Geometry: see drawing. Coordinates: mm, zero at the bounding-box minimum. A direction names the side the tool comes from. Coordinates: 2 decimals unless noted, no trailing zeros. Loops run counter-clockwise (first coordinate to the right, second up) from the corner with the lowest first, then second, coordinate; pieces in that order, holes last.
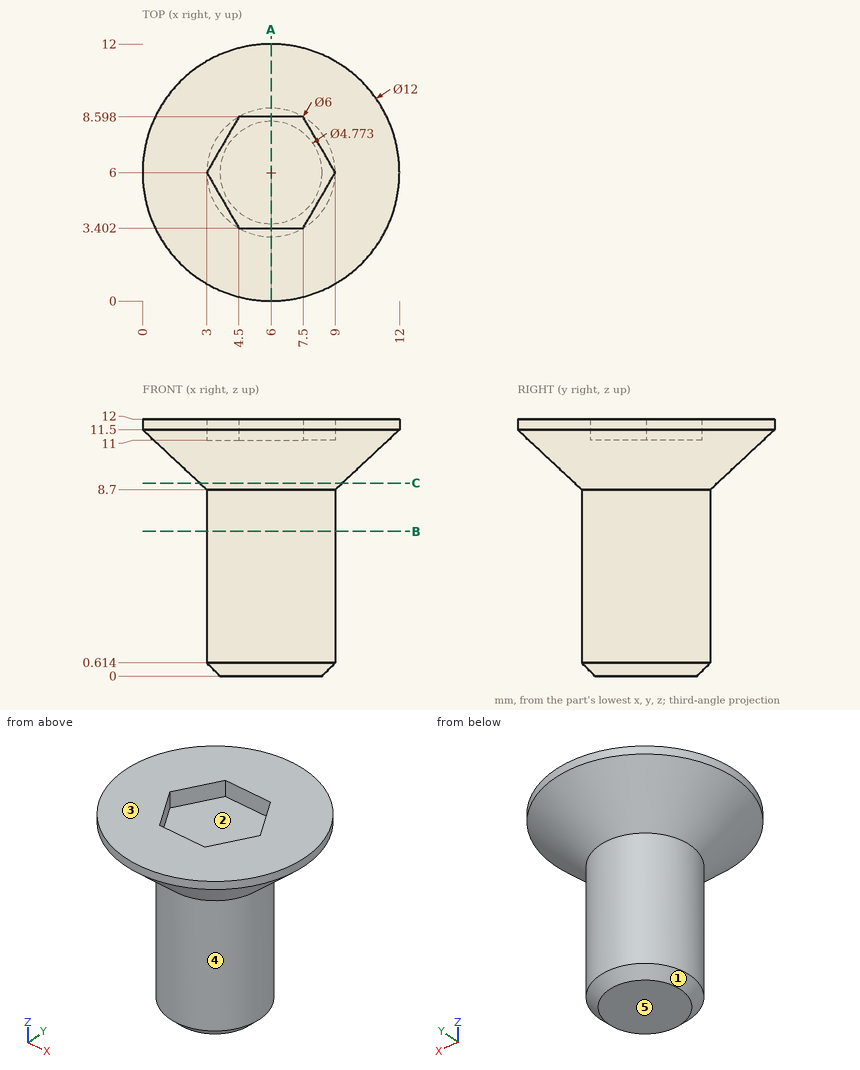
Item 1: Line query: L1, parallel to Y at x = 6, z = 1; L2, parallel to X at y = 5, z = 8; L3, parallel to X at y = 2.5, z = 10.25 (1 decimal). Output: solid intervals per line, ascending.
Result:
L1: y = 3 to 9
L2: x = 3.17 to 8.83
L3: x = 2.9 to 9.1
Item 2: Section query B-B (z = 6.75). Output: boundary loops of the cut face in (x, y), then the cut area to 3 significant figures.
Result:
outline: circle Ø6 at (6, 6)
area: 28.3 mm2
Item 3: Mould query, pull axis X, two halves, no side actions, for the marked faces 1, 2 and 3. Classes: +X half, -X half, draft (parallel to the pull), parting line (faces both ways), or undercut.
Result:
face 1: parting line
face 2: undercut
face 3: draft
Item 4: Section query A-A (x = 6). Output: boundary loops of the cut face in (y, z).
Result:
outline: (0, 11.5) - (3, 8.7) - (3, 0.61) - (3.61, 0) - (8.39, 0) - (9, 0.61) - (9, 8.7) - (12, 11.5) - (12, 12) - (8.6, 12) - (8.6, 11) - (3.4, 11) - (3.4, 12) - (0, 12) - close
Item 5: Contact query for flat-ended pins moving along their axis: P1, Ø1, axis at x = 1.5, z = 4.5, coming from the -Y side; P2, Ø4, axis at x = 7, y = 7.5, coming from the +Z side; P3, Ø1.6, axis at x = 5, y = 7, coming from the +Z side; P4, Ø5, axis at x = 8, z = 5.5, coming from the +Y side. Output: stop coordinate, or through.
Result:
P1: passes through
P2: stops at z = 12
P3: stops at z = 11
P4: stops at y = 9
Item 6: Reachability of the marked faces 4 and 5 from +Z, -Z, +X, -X, +Y, -Y: full face, straight path, thin tool, end or side. Return the list, or none.
Result:
face 4: -Z
face 5: -Z, +X, -X, +Y, -Y
Item 7: Section query C-C (z = 9). Output: boundary loops of the cut face in (x, y).
Result:
outline: circle Ø6.64 at (6, 6)
